from build123d import *

# Parameters (mm, degrees)
SKETCH_1_W          = 690
SKETCH_1_H          = 450
EXTRUDE_1_DEPTH     = 10
SKETCH_2_R          = 13.5
CUT_EXTRUDE_1_DEPTH = 10


with BuildPart() as part:
    # 草图1 → 凸台-拉伸1 (new body)
    with BuildSketch(Plane.XY):
        Rectangle(SKETCH_1_W, SKETCH_1_H)
    extrude(amount=EXTRUDE_1_DEPTH)

    # 草图2 → 切除-拉伸1 (cut)
    with BuildSketch(Plane.XY.offset(10)):
        Polygon((-345, 225), (-345, 120), (5, 225), align=None)
        Polygon((345, 225), (5, 225), (345, 20), align=None)
        Polygon((345, -20), (5, -225), (345, -225), align=None)
        Polygon((5, -225), (-345, -120), (-345, -225), align=None)
        with Locations((-305, -85)):
            Circle(SKETCH_2_R)
        with Locations((-305, 85)):
            Circle(SKETCH_2_R)
    extrude(amount=-CUT_EXTRUDE_1_DEPTH, mode=Mode.SUBTRACT)


solid = part.part
CAD build for the part. Positions are in the model's coordinates, mm. Round coordinates to 2 decimals unless told otherwise and drop trailing zeros. Loops run counter-clockwise (first coordinate to the right, second up) from the corner with the lowest first, then second, coordinate; pieces in that order, holes last.
(1) Cut at D-D (x = -150). Give the cut face in (y, z), plus the area to 3 significant figures.
(2) Two-plate mould, pull along Y, no slides. Class faces 1 (the flat face through (-81, 3, 0)), 2 (the cylindrical face through (-292.53, 79.83, 5.07)), 3 (the flat face through (177.38, -121.065, 5.07)), 4 (the flat face through (172.62, 123.935, 5.07)): +Y half, -Y half, draft (parallel to the pull), parting line (faces both ways), or undercut.
(3) Drop flat-ended pins along their axis: pin 1 (4 mm diameter, centred on x = -133, y = -129.5, fed in from -Z); pin 2 (1.5 mm diameter, centred on x = -269.5, z = 2.5, fed in from +Y) (3 decimals); pin 3 (5 mm diameter, centred on x = 115.5, z = 8.5, fed in from +Y); pin 4 (1 mm diameter, centred on y = 48.5, z = 1.5, fed in from +X). Give the stop position or say it passes through.
(4) Cut at C-C (y = 85). Give the cut face in (x, z).
(5) Cut at A-A (x = -305). Give the cut face in (y, z), plus the area to 3 significant figures.
(6) Wall check: line 1 along Y through (x, z) = (-305, 3.75); line 2 along Y through (x, z) = (112.5, 6); line 3 along X through (y, z) = (116.5, 3.75). Give the ranges that are in metal, low to high.
(7) Cut at B-B (z = 4.5). Give the cut face in (x, y), plus the area to 3 significant figures.
Findings below:
1. outline: (-178.5, 0) - (178.5, 0) - (178.5, 10) - (-178.5, 10) - close
1. area: 3,570 mm2
2. face 1: draft
2. face 2: undercut
2. face 3: -Y half
2. face 4: +Y half
3. pin 1: stops at z = 0
3. pin 2: stops at y = 142.875
3. pin 3: stops at y = 159.88
3. pin 4: stops at x = 298.56
4. outline: (-345, 0) - (-318.5, 0) - (-318.5, 10) - (-345, 10) - close; (-291.5, 0) - (237.2, 0) - (237.2, 10) - (-291.5, 10) - close
5. outline: (-132, 0) - (-98.5, 0) - (-98.5, 10) - (-132, 10) - close; (-71.5, 0) - (71.5, 0) - (71.5, 10) - (-71.5, 10) - close; (98.5, 0) - (132, 0) - (132, 10) - (98.5, 10) - close
5. area: 2,100 mm2
6. line 1: y = -132 to -98.5, -71.5 to 71.5, 98.5 to 132
6. line 2: y = -160.18 to 160.18
6. line 3: x = -345 to 184.95
7. outline: (-345, -120) - (5, -225) - (345, -20) - (345, 20) - (5, 225) - (-345, 120) - close; hole circle Ø27 at (-305, -85); hole circle Ø27 at (-305, 85)
7. area: 203,000 mm2
